Source: CAD feature listing. Evaluate the final solid. Frame: model axes, mm. Give positions to 0.01 mm unless a question says otherwise; leave off trailing zeros. Loops run counter-clockwise (first coordinate to the right, second up) from the corner with the lowest first, then second, coordinate; pieces in that order, holes last. Notation, with made-up numbers: (37, 40.25) -> (89, 40.25) arc R29 cw to (89, 64.25) -> close; hole circle Ø2 at (27.25, 26.5). An arc over 180 degrees is marked (long way). Return JSON: item names as keys, results as strings. Group by question number.
```python
from build123d import *

# Parameters (mm, degrees)
SKETCH1_W           = 19
SKETCH1_H           = 19
BOSS_EXTRUDE1_DEPTH = 115.75
CHAMFER1_SIZE       = 12


with BuildPart() as part:
    # Sketch1 → Boss-Extrude1 (new, symmetric)
    with BuildSketch(Plane.XY):
        Rectangle(SKETCH1_W, SKETCH1_H)
    extrude(amount=BOSS_EXTRUDE1_DEPTH, both=True)

    # Chamfer1
    chamfer1_edges = [part.edges().sort_by_distance(p)[0] for p in [
        (0, -9.5, 115.75),
    ]]
    chamfer(chamfer1_edges, length=CHAMFER1_SIZE)


solid = part.part
```
1) Material intervals for line 1 (Z direction, x = 2.25, y = -2.25); line 2 (Z direction, x = 4, y = -6.5), sorted ascending.
2) Contact query for a flat-ended pin moving along its axis: P1, Ø8, axis at x = 3.5, y = -2.5, coming from the +Z side. Output: stop coordinate, or through.
3) Cut plane B-B on y = -1.25. Return loops of the section in (x, z), then the cut area to 3 significant figures.
4) Cut plane A-A on x = 4.5. Return loops of the section in (y, z), then the cut area to 3 significant figures.
Calculated:
{
 "1": {"line 1": "-115.75 to 111", "line 2": "-115.75 to 106.75"},
 "2": {"P1": "z = 114.75"},
 "3": {"outline": "(-9.5, -115.75) -> (9.5, -115.75) -> (9.5, 112) -> (-9.5, 112) -> close", "area": "4,330 mm2"},
 "4": {"outline": "(-9.5, -115.75) -> (9.5, -115.75) -> (9.5, 115.75) -> (2.5, 115.75) -> (-9.5, 103.75) -> close", "area": "4,330 mm2"}
}
